from build123d import *

# Parameters (mm, degrees)
SKETCH_1_W                = 30
SKETCH_1_H                = 580
EXTRUDE_1_DEPTH           = 48
SKETCH_2_W                = 20
SKETCH_2_H                = 580
CUT_EXTRUDE_1_DEPTH       = 2
PATTERN_LINEAR_1_COUNT    = 10
PATTERN_LINEAR_1_PITCH    = 60
HOLE_WIZARD_1_D           = 6.6
HOLE_WIZARD_1_CBORE_D     = 11
HOLE_WIZARD_1_CBORE_DEPTH = 6.8
PATTERN_LINEAR_2_COUNT    = 5
PATTERN_LINEAR_2_PITCH    = 120


with BuildPart() as part:
    # 草图1 → 凸台-拉伸1 (new body)
    with BuildSketch(Plane.XY):
        Rectangle(SKETCH_1_W, SKETCH_1_H)
    extrude(amount=EXTRUDE_1_DEPTH)

    # 草图2 → 切除-拉伸1 (cut)
    with BuildSketch(Plane(origin=(0, 0, 0), x_dir=(-1, 0, 0), z_dir=(0, 0, -1))):
        with Locations((5, 0)):
            Rectangle(SKETCH_2_W, SKETCH_2_H)
    extrude(amount=-CUT_EXTRUDE_1_DEPTH, mode=Mode.SUBTRACT)

    # 草图4 → M5 螺纹孔1 (revolve, cut)
    with BuildSketch(Plane(origin=(-5, 270, 2), x_dir=(0, 1, 0), z_dir=(1, 0, 0))):
        Polygon((0, 0), (0, 13.6618073), (2.1, 12.4), (2.1, 0), align=None)
    hole_wizard_m5_1 = revolve(axis=Axis((-5, 270, -4.35), (0, 0, 1)), mode=Mode.SUBTRACT)

    # 阵列(线性)1: M5 螺纹孔1 ×10
    with Locations(*[(0, -i * PATTERN_LINEAR_1_PITCH, 0) for i in range(1, PATTERN_LINEAR_1_COUNT)]):
        add(hole_wizard_m5_1, mode=Mode.SUBTRACT)

    # 打孔尺寸(%根据)内六角圆柱头螺钉的类型1 (through all)
    with Locations(Plane(origin=(0, 0, 2), x_dir=(-1, 0, 0), z_dir=(0, 0, -1))):
        with Locations((5, 240)):
            hole_wizard_1 = CounterBoreHole(HOLE_WIZARD_1_D / 2, HOLE_WIZARD_1_CBORE_D / 2, HOLE_WIZARD_1_CBORE_DEPTH)

    # 阵列(线性)2: 打孔尺寸(%根据)内六角圆柱头螺钉的类型1 ×5
    with Locations(*[(0, -i * PATTERN_LINEAR_2_PITCH, 0) for i in range(1, PATTERN_LINEAR_2_COUNT)]):
        add(hole_wizard_1, mode=Mode.SUBTRACT)


solid = part.part
Can you work these out from the model? Positions are in its coordinate system, mm. A direction names the side the tool comes from. Coordinates: 2 decimals unless noted, no trailing zeros. Order: outer loops, then holes, each group sorted by start corner. A loop starts at its lowest first (then second) coordinate and runs counter-clockwise, first axis right, second up. Notation, with made-up numbers: M 71,-40 L 121,-40 A17 ccw 121,-18 Z; hole C -3.75,50 d7. An arc over 180 degrees is marked long. Write item = value, one per line.
(1) Suppose I cut it at A-A on y = 57. Please give me the cut outline in (x, z).
Results are:
outline = M -15,2 L 5,2 L 5,0 L 15,0 L 15,48 L -15,48 Z
(2) For pin 1 Ø10.5 at (x, y) = (-5, 0) entering from +Z; pin 2 Ø5 at (x, y) = (-5, -90) entering from -Z; pin 3 Ø4 at (x, y) = (-5, -120) entering from -Z; pin 4 Ø9 at (x, y) = (-5, 0) entering from -Z, each with a flat end and sliding along its axis, tell me the tip position at first contact or that it passes through.
Results are:
pin_1 = 48
pin_2 = 2
pin_3 = through
pin_4 = 8.8
(3) I need wall thicknesses on line 1 along Y through (x, z) = (-5, 38); line 2 along X through (y, z) = (240, 36); line 3 along X through (y, z) = (150, 9.25). Which ranges of each line are inside material? Lowest first, please. Write a range as [from, to].
Results are:
line_1 = [-290, -243.3], [-236.7, -123.3], [-116.7, -3.3], [3.3, 116.7], [123.3, 236.7], [243.3, 290]
line_2 = [-15, -8.3], [-1.7, 15]
line_3 = [-15, -7.1], [-2.9, 15]
(4) If we mould it in two halves opening along Y, with no side actions, what happens to faces 1 (the face through (-10.08, -2.11, 5.35)), 2 (the face through (0, 290, 24)), 3 (the face through (-15, -4, 25))? For each: pulls with the +Y half, pulls with the -Y half, needs draft (parallel to the pull), parting line crosses it, or undercut.
Results are:
face_1 = undercut
face_2 = pulls with the +Y half
face_3 = needs draft
(5) For faces 4 (the face through (-9, 240, 8.8)), 5 (the face through (0, 4, 48)), 6 (the face through (0, 4, 2)), which set-ups out of +Z, -Z, +X, -X, +Y, -Y let a thin tool reach every point of the face, with its end or its side?
Results are:
face_4 = -Z
face_5 = +Z, +X, -X, +Y, -Y
face_6 = -Z, -X, +Y, -Y
